Source: three-view drawing plus pictorial views. Frame: mm from the lowest corner of the part. Give positions to 0.01 mm unless a question says otherwise; leave off trailing zeros. Write each loop counter-clockwise with the first axis right and the second up, starting at its lowest first coordinate (ties: lowest second). Pieces come first, ordered by that corner, then holes. Notation, with made-up numbers: (73, -4.75) -> (123, -4.75) arc R27 cw to (123, 15.25) -> close; hole circle Ø11 at (50.5, 35.25). An arc over 180 degrees is marked (long way). Answer in a Markdown table with one row per item. Add a question column.
Item 1: Material intervals for probe 1 along Y at (x, z) = (11, 24.5); probe 2 along Z at (x, y) = (47, 21), sorted ascending. Write a range as from..to.
Item 2: Section query C-C on z = 11.5. Output: boundary loops of the cut face in (x, y), plus the area to 3 significant figures.
Item 3: Section query D-D on y = 14. Output: boundary loops of the cut face in (x, z), plus the area to 3 significant figures.
Item 4: First-contact query: P1, Ø1.5, axis at y = 7.5, z = 7, coming from the -X side. Flat tip, straight axial feed; report the tip coordinate or a pass-through.
Item 5: Draft query along X for the marked faces 1, 2, 3 and 4. Return one class per face: +X half, -X half, draft (parallel to the pull), parting line (faces both ways), or undercut.
Item 6: Section query A-A on y = 8. Output: boundary loops of the cut face in (x, z).
Item 7: Section query B-B on x = 62.5. Output: boundary loops of the cut face in (y, z).
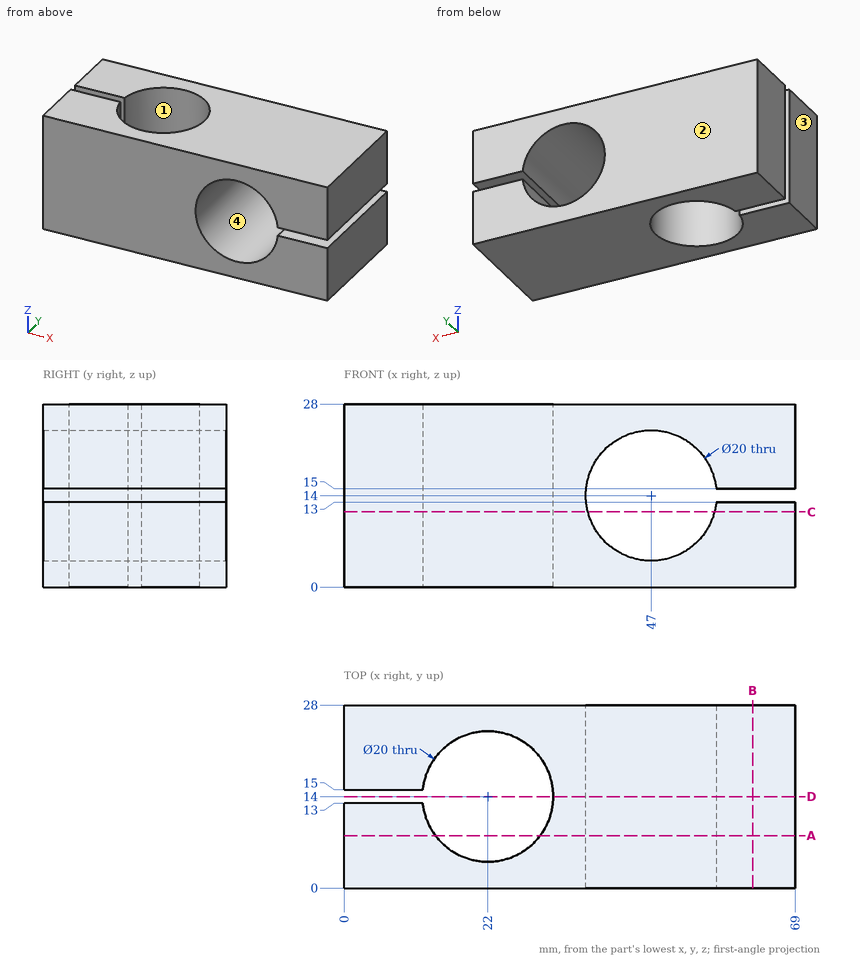
Findings below:
| question | item | result |
|---|---|---|
| 1 | probe 1 | y = 0..13, 15..28 |
| 1 | probe 2 | z = 0..4, 24..28 |
| 2 | outline | (0, 0) -> (37.32, 0) -> (37.32, 28) -> (0, 28) -> (0, 15) -> (12.05, 15) arc R10 cw (long way) to (12.05, 13) -> (0, 13) -> close; (56.68, 0) -> (69, 0) -> (69, 28) -> (56.68, 28) -> close |
| 2 | area | 1,050 mm^2 |
| 3 | outline | (32, 0) -> (69, 0) -> (69, 13) -> (56.95, 13) arc R10 cw (long way) to (56.95, 15) -> (69, 15) -> (69, 28) -> (32, 28) -> close |
| 3 | area | 698 mm^2 |
| 4 | P1 | stops at x = 0 |
| 5 | face 1 | undercut |
| 5 | face 2 | draft |
| 5 | face 3 | -X half |
| 5 | face 4 | undercut |
| 6 | outline | (0, 0) -> (14, 0) -> (14, 28) -> (0, 28) -> close; (30, 0) -> (69, 0) -> (69, 13) -> (56.95, 13) arc R10 cw (long way) to (56.95, 15) -> (69, 15) -> (69, 28) -> (30, 28) -> close |
| 7 | outline | (0, 0) -> (28, 0) -> (28, 13) -> (0, 13) -> close; (0, 15) -> (28, 15) -> (28, 28) -> (0, 28) -> close |
